from build123d import *

# Parameters (mm, degrees)
BASE_PLATE_SKETCH_R           = 4
BASE_PLATE_DEPTH              = 5
SIDE_WALL_SKETCH_W            = 5
SIDE_WALL_SKETCH_H            = 40
SIDE_WALL_DEPTH               = 20
SIDE_WALL_TAPER_CUT_DEPTH     = 20
BACK_WALL_SKETCH_W            = 75
BACK_WALL_SKETCH_H            = 5
BACK_WALL_DEPTH               = 30
BACK_WALL_CORNER_RADIUS_DEPTH = 30


with BuildPart() as part:
    # Base Plate Sketch → Base Plate (new body)
    with BuildSketch(Plane(origin=(0, 0, 0), x_dir=(1, 0, 0), z_dir=(0, 1, 0))):
        Polygon((0, 0), (75, 0), (75, -25), (60, -40), (0, -40), align=None)
        with Locations(Location((20, -25, 0), (0, 0, 270))):
            Circle(BASE_PLATE_SKETCH_R, mode=Mode.SUBTRACT)
        with Locations(Location((55, -25, 0), (0, 0, 270))):
            Circle(BASE_PLATE_SKETCH_R, mode=Mode.SUBTRACT)
    extrude(amount=BASE_PLATE_DEPTH)

    # Side Wall Sketch → Side Wall (add)
    with BuildSketch(Plane(origin=(0, 5, 0), x_dir=(1, 0, 0), z_dir=(0, 1, 0))):
        with Locations((2.5, -20)):
            Rectangle(SIDE_WALL_SKETCH_W, SIDE_WALL_SKETCH_H)
    extrude(amount=SIDE_WALL_DEPTH)

    # Side Wall Taper Sketch → Side Wall Taper Cut (cut)
    with BuildSketch(Plane(origin=(5, 0, 0), x_dir=(0, 0, -1), z_dir=(1, 0, 0))):
        Polygon((-19, 20), (-40, 12), (-40, 25), (0, 25), (0, 20), align=None)
    extrude(amount=-SIDE_WALL_TAPER_CUT_DEPTH, mode=Mode.SUBTRACT)

    # Back Wall Sketch → Back Wall (add)
    with BuildSketch(Plane(origin=(0, 5, 0), x_dir=(1, 0, 0), z_dir=(0, 1, 0))):
        with Locations((37.5, -2.5)):
            Rectangle(BACK_WALL_SKETCH_W, BACK_WALL_SKETCH_H)
    extrude(amount=BACK_WALL_DEPTH)

    # Back Wall Corner Radius Sketch → Back Wall Corner Radius (cut)
    with BuildSketch(Plane.XY.offset(5)):
        with BuildLine():
            Line((50, 35), (75, 35))
            Line((75, 35), (75, 10))
            ThreePointArc((75, 10), (67.67766953, 27.67766953), (50, 35))
        make_face()
    extrude(amount=-BACK_WALL_CORNER_RADIUS_DEPTH, mode=Mode.SUBTRACT)


solid = part.part
The listing builds one solid part. Answer for the finished solid, in the listing's coordinates (mm). A direction names the side the tool comes from. Round coordinates to 2 decimals unless told otherwise and drop trailing zeros. Write each loop counter-clockwise with the first axis right and the second up, starting at its lowest first coordinate (ties: lowest second). Pieces come first, ordered by that corner, then holes. Notation, with made-up numbers: (-19, -17) - (10, -17) arc R22 cw to (10, 13) - close; hole circle Ø5 at (72.5, 80). An arc over 180 degrees is marked (long way). Use one line per item in the form item = value. Start each with the question number.
Item 1: A cutting plane is placed at D-D (x = 55). Write down the section's boundary in (y, z).
Item 2: Determine the mould class of faces 1 (the cylindrical face through (51.095, 2.465, 24.133)), 2 (the flat face through (75, 4, 10)), 3 (the flat face through (38, 0, 20)) for opening direction X: +X half, -X half, draft (parallel to the pull), parting line (faces both ways), or undercut.
Item 3: A tool of negligible diameter and unlimited length cuts with its end or side. For faces 4 (the flat face through (3, 20, 12)), 5 (the flat face through (0, 9, 16)), 6 (the flat face through (5, 11, 23)), from which of +Z, -Z, +X, -X, +Y, -Y can it reach the whole face along a straight path? Write none if from no direction.
Item 4: A cutting plane is placed at A-A (x = 20). Write down the section's boundary in (y, z).
Item 5: A cutting plane is placed at C-C (y = 18.5). Write down the section's boundary in (x, z), plus the area to 3 significant figures.
Item 6: Flat-ended cylindrical pins translate along their axes: pin 1 Ø3 at (x, z) = (25.5, 7) entering from +Y; pin 2 Ø5 at (x, z) = (18.5, 7) entering from -Y; pin 3 Ø7.5 at (y, z) = (15, 21) entering from +X; pin 4 Ø4 at (x, z) = (3.5, 12.5) entering from +Y. Find the tip coordinate at first contact, or state that the pin passes through.
Item 7: A cutting plane is placed at B-B (x = 44.5). Write down the section's boundary in (y, z), plus the area to 3 significant figures.
Item 8: Find the intervals of material crossed by line 1 (X direction, y = 3.8, z = 25); line 2 (Z direction, x = 65, y = 16), in increasing order. Write a range as [from, to].
The answers:
q1.outline = (0, 0) - (34.49, 0) - (34.49, 5) - (5, 5) - (5, 21) - (0, 21) - close; (0, 29) - (5, 29) - (5, 40) - (0, 40) - close
q2.face_1 = undercut
q2.face_2 = +X half
q2.face_3 = draft
q3.face_4 = +Z, +X, -X, +Y
q3.face_5 = +Z, -Z, -X, +Y, -Y
q3.face_6 = +Z, +X, +Y
q4.outline = (0, 0) - (35, 0) - (35, 5) - (5, 5) - (5, 21) - (0, 21) - close; (0, 29) - (5, 29) - (5, 40) - (0, 40) - close
q5.outline = (0, 0) - (73.51, 0) - (73.51, 5) - (5, 5) - (5, 22.94) - (0, 22.94) - close
q5.area = 457 mm^2
q6.pin_1 = 5
q6.pin_2 = 0
q6.pin_3 = 5
q6.pin_4 = 20
q7.outline = (0, 0) - (35, 0) - (35, 5) - (5, 5) - (5, 40) - (0, 40) - close
q7.area = 350 mm^2
q8.line_1 = [0, 16], [24, 51], [59, 75]
q8.line_2 = [0, 5]
